Could you check a few things on this drawing? It's one solid part, dimensions in mm from its lowest x, y, z. A direction names the side the tool comes from. Give positions to 0.01 mm unless a question says otherwise; leave off trailing zeros. Order: outer loops, then holes, each group sorted by start corner. A loop starts at its lowest first (then second) coordinate and runs counter-clockwise, first axis right, second up.
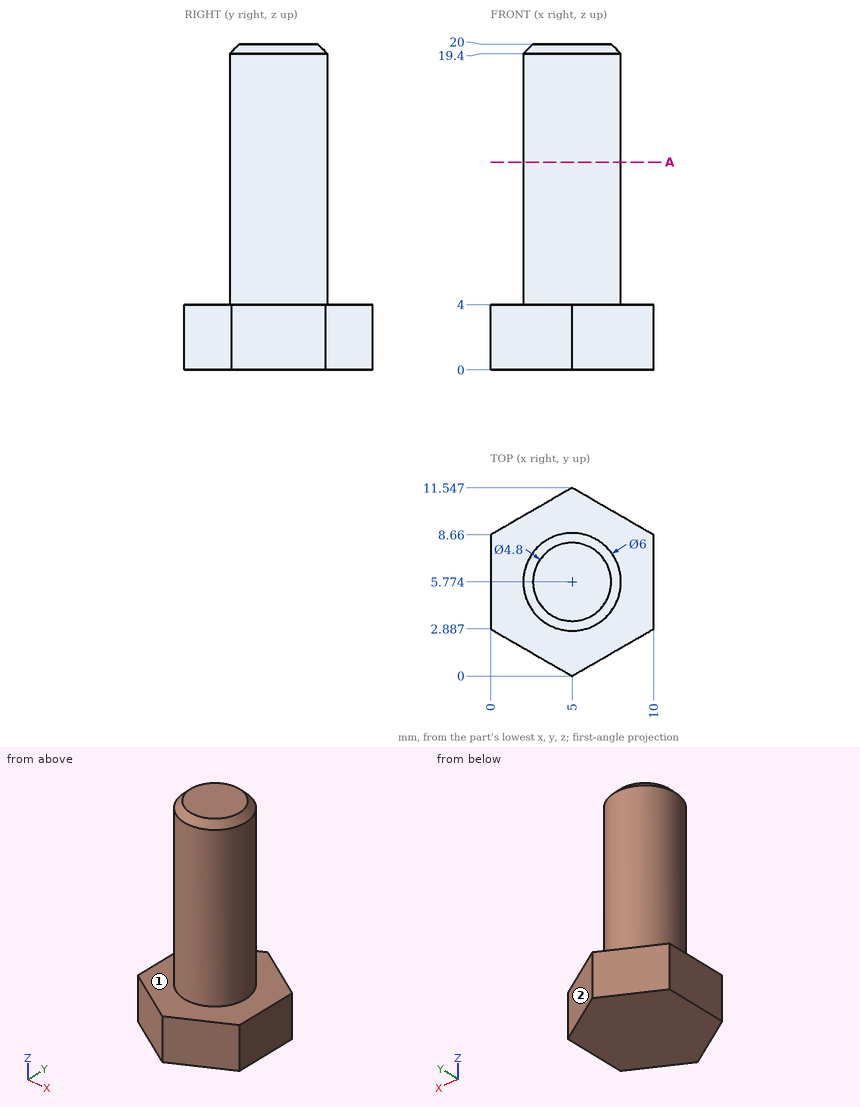
Item 1: Imagine slicing it at A-A on z = 12.75. List the corners of the cut face in (x, y) for me.
Findings:
outline: circle Ø6 at (5, 5.77)
Item 2: For pin 1 (6 mm diameter, centred on x = 4.5, z = 10.5, fed in from +Y); pin 2 (1.5 mm diameter, centred on x = 3, z = 17.5, fed in from -Y); pin 3 (5 mm diameter, centred on y = 3.5, z = 11.5, fed in from -X), each with a flat end and sliding along its axis, tell me the tip position at first contact or that it passes through.
Findings:
pin 1: stops at y = 8.77
pin 2: stops at y = 3.05
pin 3: stops at x = 2
Item 3: Please list where these lines run through material, in increasing order: line 1 along Z through (x, y) = (5.25, 1.5); line 2 along X through (y, z) = (6.75, 10) (1 decimal); line 3 along Y through (x, z) = (4.5, 6.75) (1 decimal).
Findings:
line 1: z = 0 to 4
line 2: x = 2.2 to 7.8
line 3: y = 2.8 to 8.7
Item 4: For the marked faces 1 and 2, which set-ups out of +Z, -Z, +X, -X, +Y, -Y let a thin tool reach every point of the face, with its end or its side?
Findings:
face 1: +Z
face 2: +Z, -Z, +X, +Y
